Source: CAD feature listing. Evaluate the final solid. Frame: model axes, mm. A direction names the side the tool comes from. Give positions to 0.01 mm unless a question says otherwise; leave off trailing zeros. Loops run counter-clockwise (first coordinate to the right, second up) from the corner with the lowest first, then second, coordinate; pieces in that order, holes last. Notation, with made-up numbers: M 76.5,-25 L 114.5,-25 A12 cw 114.5,-2 Z; hole C -19.75,66 d10. An arc over 180 degrees is marked long. Answer in a Markdown table with one row per item.
```python
from build123d import *

# Parameters (mm, degrees)
CHAMFER1_SIZE = 0.5


with BuildPart() as part:
    # Sketch1 → Revolve1 (revolve)
    with BuildSketch(Plane.XY, mode=Mode.PRIVATE) as revolve1_sk:
        Polygon((-24, 12), (-24, 10), (24, 10), (24, 12), (30, 12), (30, 15), (15, 15), (15, 14), (-15, 14), (-15, 15), (-30, 15), (-30, 12), align=None)
    revolve(revolve1_sk.sketch.rotate(Axis((48.533661203, 0, 0), (-1, 0, 0)), 90), axis=Axis((48.533661203, 0, 0), (-1, 0, 0)))

    # Chamfer1
    chamfer1_edges = [part.edges().sort_by_distance(p)[0] for p in [
        (30, 0, 12),
        (-30, 0, 12),
        (-30, 0, 15),
        (-15, 0, 15),
        (15, 0, 15),
        (30, 0, 15),
    ]]
    chamfer(chamfer1_edges, length=CHAMFER1_SIZE)


solid = part.part
```
Q1. Contact query for flat-ended pins moving along their axis: pin 1 Ø2 at (x, z) = (-19.5, 6) entering from -Y; pin 2 Ø3 at (x, y) = (-14, 12) entering from -Z; pin 3 Ø4 at (x, y) = (22, -6.5) entering from +Z. Output: stop coordinate, or through.
Values follow:
| item | result |
|---|---|
| pin 1 | y = -14.14 |
| pin 2 | z = -9.64 |
| pin 3 | z = 14.31 |
Q2. Ray query, probe 1 along Y at (x, z) = (25.4, 0); probe 2 along Y at (x, z) = (-3.5, 0); probe 3 along X at (y, z) = (5.25, -9.5). Return the intervals inside material, ascending. Write a range as from..to.
Values follow:
| item | result |
|---|---|
| probe 1 | -15..-12, 12..15 |
| probe 2 | -14..-10, 10..14 |
| probe 3 | -24..24 |
Q3. Mould query, pull axis X, two halves, no side actions, for faces 3 (the flat face through (-30, -7, 11)), 4 (the cylindrical face through (26.788, -3.604, -11.446)), 5 (the cylindrical face through (-0.2, 12.4, -6.5)), 6 (the flat face through (24, -9, -5)). Classes: +X half, -X half, draft (parallel to the pull), parting line (faces both ways), or undercut.
Values follow:
| item | result |
|---|---|
| face 3 | -X half |
| face 4 | draft |
| face 5 | undercut |
| face 6 | +X half |
Q4. Section query B-B (x = -12.5). Output: boundary loops of the cut face in (y, z).
Values follow:
| item | result |
|---|---|
| outline | C 0,0 d28; hole C 0,0 d20 |
Q5. Section query A-A (x = 25). Output: boundary loops of the cut face in (y, z).
Values follow:
| item | result |
|---|---|
| outline | C 0,0 d30; hole C 0,0 d24 |
Q6. Reachability of faces 1 (the flat face through (-24, -9, 5)), 2 (the flat face through (30, -7, -11)) from +Z, -Z, +X, -X, +Y, -Y: full face, straight path, thin tool, end or side. Return the list, or none.
Values follow:
| item | result |
|---|---|
| face 1 | -X |
| face 2 | +Z, -Z, +X, +Y, -Y |
